```python
from build123d import *

# Parameters (mm, degrees)
SKETCH1_R      = 13.5
EXTRUDE1_DEPTH = 2


with BuildPart() as part:
    # Sketch1 → Extrude1 (new, symmetric)
    with BuildSketch(Plane(origin=(0, 0, 0), x_dir=(1, 0, 0), z_dir=(0, 1, 0))):
        with BuildLine():
            Line((-62, 26), (0, 26))
            ThreePointArc((0, 26), (26, 0), (0, -26))
            Line((0, -26), (-62, -26))
            ThreePointArc((-62, -26), (-88, 0), (-62, 26))
        make_face()
        with Locations(Location((0, 0, 0), (0, 0, 270))):
            Circle(SKETCH1_R, mode=Mode.SUBTRACT)
        with Locations(Location((-62, 0, 0), (0, 0, 270))):
            Circle(SKETCH1_R, mode=Mode.SUBTRACT)
    extrude(amount=EXTRUDE1_DEPTH, both=True)


solid = part.part
```
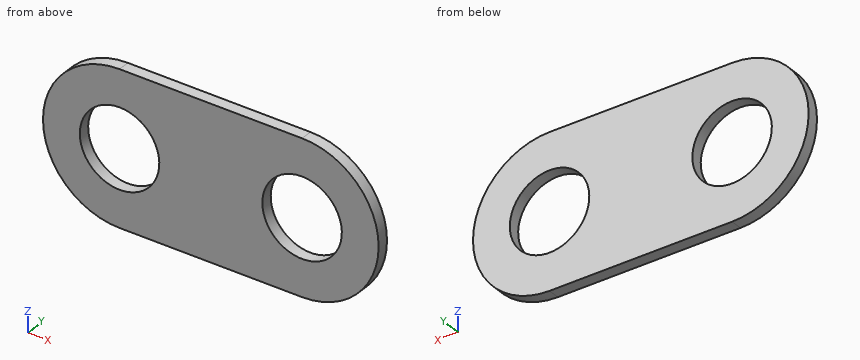
The listing builds one solid part. Answer for the finished solid, in the listing's coordinates (mm). Coordinates: 2 decimals unless noted, no trailing zeros. Write each loop counter-clockwise with the first axis right and the second up, starting at its lowest first coordinate (ties: lowest second). Pieces come first, ordered by that corner, then holes. Notation, with made-up numbers: (-9, 30) - (5, 30) arc R26 cw to (5, 50) - close; hole circle Ø2 at (24.25, -14). An arc over 180 degrees is marked (long way). Return JSON: item names as keys, results as strings. Group by question number.
Q1. The part is cut by section C-C on y = -0.1. Write down the section's boundary in (x, z).
Q2. The part is cut by section A-A on z = 0. Write down the section's boundary in (x, y), and give its area (3 significant figures).
Q3. The part is cut by section B-B on x = -5. Write down the section's boundary in (y, z).
Q4. A flat-ended cylindrical pin translates along its axis: pin 1 Ø1 at (y, z) = (-0.5, -8) entering from -X. Find the tip coordinate at first contact, or state that the pin passes through.
Q5. The part is cut by section D-D on x = 6.5. Write down the section's boundary in (y, z), and give its area (3 significant figures).
Q6. Find the intervals of material crossed by line 1 along X through (y, z) = (0.05, 0); line 2 along X through (y, z) = (0.4, -3); line 3 along Z through (x, y) = (-1.5, 1.3), in increasing order. Write a range as [from, to].
Evaluation:
{
 "1": {"outline": "(-62, -26) - (0, -26) arc R26 ccw to (0, 26) - (-62, 26) arc R26 ccw to start; hole circle Ø27 at (-62, 0); hole circle Ø27 at (0, 0)"},
 "2": {"outline": "(-88, -2) - (-75.5, -2) - (-75.5, 2) - (-88, 2) - close; (-48.5, -2) - (-13.5, -2) - (-13.5, 2) - (-48.5, 2) - close; (13.5, -2) - (26, -2) - (26, 2) - (13.5, 2) - close", "area": "240 mm2"},
 "3": {"outline": "(-2, -26) - (2, -26) - (2, -12.54) - (-2, -12.54) - close; (-2, 12.54) - (2, 12.54) - (2, 26) - (-2, 26) - close"},
 "4": {"pin 1": "stops at x = -86.89"},
 "5": {"outline": "(-2, -25.17) - (2, -25.17) - (2, -11.83) - (-2, -11.83) - close; (-2, 11.83) - (2, 11.83) - (2, 25.17) - (-2, 25.17) - close", "area": "107 mm2"},
 "6": {"line 1": "x = [-88, -75.5], [-48.5, -13.5], [13.5, 26]", "line 2": "x = [-87.83, -75.16], [-48.84, -13.16], [13.16, 25.83]", "line 3": "z = [-26, -13.42], [13.42, 26]"}
}
